Could you check a few things on this model? Use its own coordinates, in mm. Give positions to 0.01 mm unless a question says otherwise; leave off trailing zeros. Loops run counter-clockwise (first coordinate to the right, second up) from the corner with the lowest first, then second, coordinate; pieces in that order, holes last. Notation, with made-up numbers: (72.25, -40) - (90.25, -40) arc R18 ccw to (90.25, -11) - close; hole circle Ø6 at (63, -20). An arc over 180 degrees is marked (long way). Write each question's results on one line, items separated by ' | '. Start each with the question number.
1) I'm going to push flat-ended pins straight in: pin 1 (1.3 mm diameter, centred on x = 0, z = 24, fed in from +Y); pin 2 (1 mm diameter, centred on y = 0.5, z = -10, fed in from -X). Where does each tip first touch, or does it pass through?
2) I want a section at B-B, the plane z = 10.5. Write out the boundary of the cut face in (x, y).
3) I want a section at A-A, the plane x = -0.3. Write out the boundary of the cut face in (y, z), and give its area (3 significant figures).
4) If I drill on probe 1 along Z at (x, y) = (-1.15, 0.6); probe 2 along Z at (x, y) = (0.65, 0.1); probe 3 along Y at (x, z) = (-0.3, 17), over which ranges is the centre line in solid material (lowest first)? Write a range as [from, to].
from build123d import *

# Parameters (mm, degrees)
BOSS_EXTRUDE1_DEPTH      = 20
BOSS_EXTRUDE1_DEPTH_BACK = 46
SKETCH1_R                = 1.5
SKETCH2_R                = 1.5
BOSS_EXTRUDE2_DEPTH      = 0.5
BOSS_EXTRUDE3_DEPTH      = 0.25


with BuildPart() as part:
    # Sketch1 → Boss-Extrude1 (new, two sides: drawn at the far end of the back side and taken through both)
    with BuildSketch(Plane.XY.offset(-BOSS_EXTRUDE1_DEPTH_BACK)):
        Circle(SKETCH1_R)
    extrude(amount=BOSS_EXTRUDE1_DEPTH + BOSS_EXTRUDE1_DEPTH_BACK)

    # Sketch2 → Boss-Extrude2 (add)
    with BuildSketch(Plane.XY.offset(20)):
        Circle(SKETCH2_R)
    extrude(amount=BOSS_EXTRUDE2_DEPTH)

    # Sketch3 → Boss-Extrude3 (add, symmetric)
    with BuildSketch(Plane(origin=(0, 0, 0), x_dir=(1, 0, 0), z_dir=(0, 1, 0))):
        with BuildLine():
            Line((0.873889529, -20.5), (-0.757865329, -20.5))
            Line((-0.757865329, -20.5), (-0.757865329, -23.138895886))
            ThreePointArc((-0.757865329, -23.138895886), (-0.472929345, -25.311777544), (0.362611115, -27.337728025))
            Line((0.362611115, -27.337728025), (0.362611115, -23.138895886))
            Line((0.362611115, -23.138895886), (0.873889529, -23.138895886))
            Line((0.873889529, -23.138895886), (0.873889529, -20.5))
        make_face()
    extrude(amount=BOSS_EXTRUDE3_DEPTH, both=True)


solid = part.part
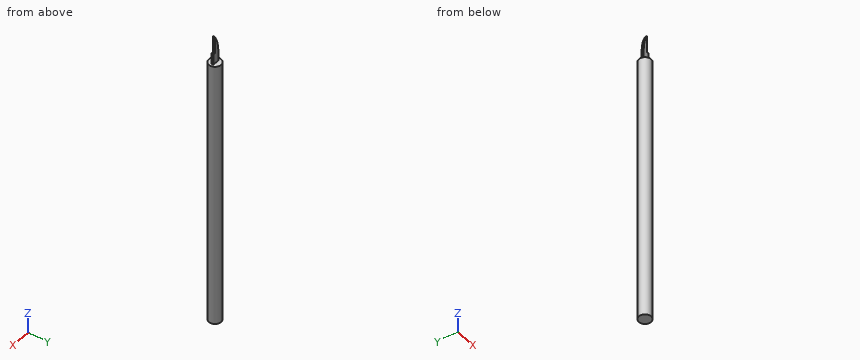
Answers:
1) pin 1: stops at y = 0.25 | pin 2: stops at x = -1.5
2) outline: circle Ø3 at (0, 0)
3) outline: (-1.47, -46) - (1.47, -46) - (1.47, 20.5) - (0.25, 20.5) - (0.25, 25.88) - (-0.25, 25.88) - (-0.25, 20.5) - (-1.47, 20.5) - close | area: 198 mm2
4) probe 1: z = [-46, 20.5] | probe 2: z = [-46, 23.14] | probe 3: y = [-1.47, 1.47]
